Source: three-view drawing plus pictorial views. Frame: mm from the lowest corner of the part. Coordinates: 2 decimals unless noted, no trailing zeros. Write each loop counter-clockwise with the first axis right and the second up, starting at its lowest first coordinate (ties: lowest second). Pieces come first, ordered by that corner, then holes. Notation, with made-up numbers: (8, 2) - (37, 2) arc R23 ccw to (37, 39) - close; hole circle Ø7 at (13, 66.25). An arc over 180 degrees is marked (long way). Put each result on its own line as item: value.
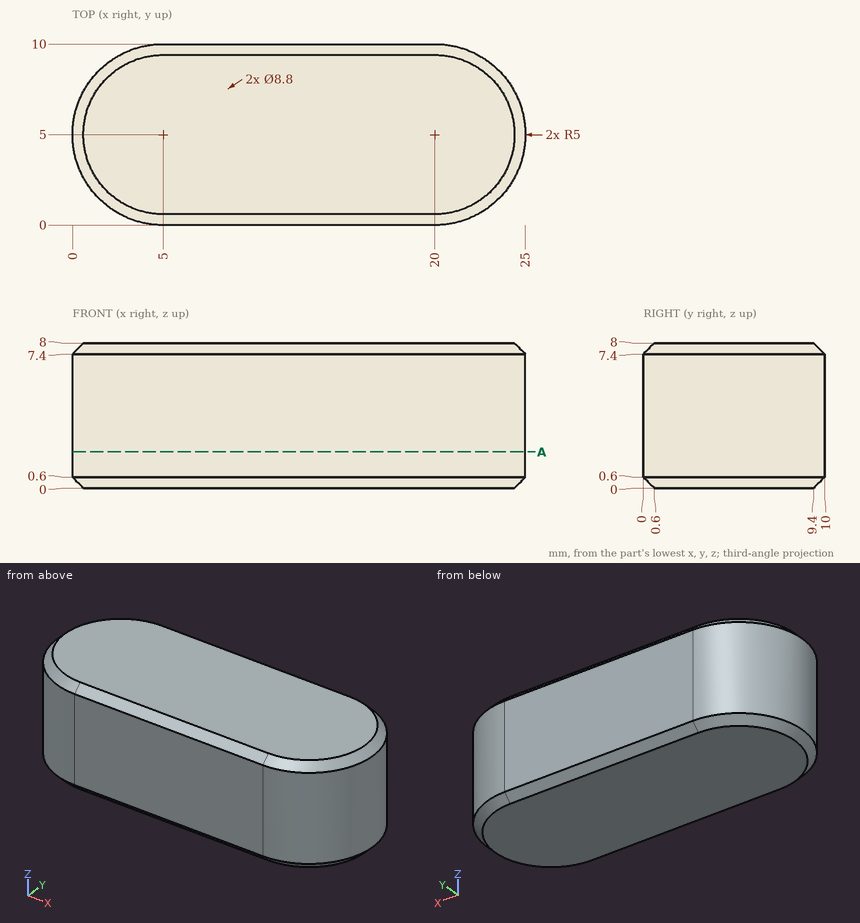
1. Ray query, probe 1 along Y at (x, z) = (22.75, 3); probe 2 along Y at (x, z) = (21.5, 0.75); probe 3 along X at (y, z) = (3, 0.75). Return the intervals inside material, ascending. Write a range as from..to.
Answer below:
probe 1: y = 0.82..9.18
probe 2: y = 0.23..9.77
probe 3: x = 0.42..24.58
2. Section query A-A (z = 2). Return loops of the section in (x, y).
Answer below:
outline: (5, 0) - (20, 0) arc R5 ccw to (20, 10) - (5, 10) arc R5 ccw to start
3. Pin query (flat end, axial travel): pin 1 Ø4 at (y, z) = (8.5, 5.5) entering from -X. Return the tip coordinate at first contact, or that it passes through.
Answer below:
pin 1: stops at x = 0.23
